from build123d import *

# Parameters (mm, degrees)
SKETCH1_W               = 1200
SKETCH1_H               = 365
BOSS_EXTRUDE1_DEPTH     = 20
CUT_EXTRUDE1_DEPTH      = 628.460158098
CUT_EXTRUDE1_DEPTH_BACK = 628.460158098
SKETCH2_R               = 20
CHAMFER1_SIZE           = 20
CHAMFER2_SIZE           = 20


with BuildPart() as part:
    # Sketch1 → Boss-Extrude1 (new body)
    with BuildSketch(Plane.XY):
        Rectangle(SKETCH1_W, SKETCH1_H)
    extrude(amount=BOSS_EXTRUDE1_DEPTH)

    # Sketch2 → Cut-Extrude1 (cut, two sides: drawn at the far end of the back side and taken through both)
    with BuildSketch(Plane.XY.offset(20).offset(-CUT_EXTRUDE1_DEPTH_BACK)):
        with Locations((-550, 102.5)):
            Circle(SKETCH2_R)
        with Locations((550, 102.5)):
            Circle(SKETCH2_R)
    extrude(amount=CUT_EXTRUDE1_DEPTH + CUT_EXTRUDE1_DEPTH_BACK, mode=Mode.SUBTRACT)

    # Chamfer1
    chamfer1_edges = [part.edges().sort_by_distance(p)[0] for p in [
        (-600, 182.5, 10),
        (600, 182.5, 10),
    ]]
    chamfer(chamfer1_edges, length=CHAMFER1_SIZE)

    # Chamfer2
    chamfer2_edges = [part.edges().sort_by_distance(p)[0] for p in [
        (600, -182.5, 10),
        (-600, -182.5, 10),
    ]]
    chamfer(chamfer2_edges, length=CHAMFER2_SIZE)


solid = part.part
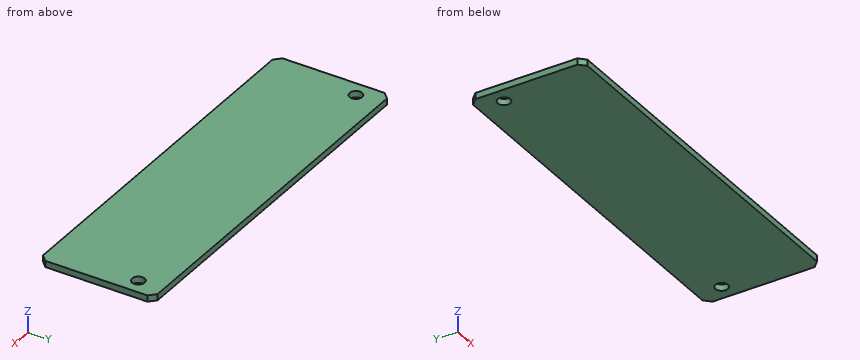
The model under review builds one solid part; all positions refer to its coordinate system, in mm. Round coordinates to 2 decimals unless told otherwise and drop trailing zeros. Loops run counter-clockwise (first coordinate to the right, second up) from the corner with the lowest first, then second, coordinate; pieces in that order, holes last. Notation, with made-up numbers: (69, 25.25) -> (80, 25.25) arc R22 cw to (80, 43.25) -> close; hole circle Ø2 at (87, -29). An arc over 180 degrees is marked (long way). Return JSON: item names as keys, results as strings.
(1) Add section B-B on x = 550. Write out the cut boundary in (y, z).
Solved:
{"outline": "(-182.5, 0) -> (82.5, 0) -> (82.5, 20) -> (-182.5, 20) -> close; (122.5, 0) -> (182.5, 0) -> (182.5, 20) -> (122.5, 20) -> close"}
(2) For line 1 (X direction, y = 102.5, z = 13.75); line 2 (Y direction, x = -550, z = 5); line 3 (X direction, y = 165, z = 19.25), list the stretches that pass through material, from the lowest coordinate up.
Solved:
{"line 1": "-600 to -570, -530 to 530, 570 to 600", "line 2": "-182.5 to 82.5, 122.5 to 182.5", "line 3": "-597.5 to 597.5"}
(3) Add section A-A on y = 102.5. Write out the cut boundary in (x, z).
Solved:
{"outline": "(-600, 0) -> (-570, 0) -> (-570, 20) -> (-600, 20) -> close; (-530, 0) -> (530, 0) -> (530, 20) -> (-530, 20) -> close; (570, 0) -> (600, 0) -> (600, 20) -> (570, 20) -> close"}
